Drawing for the job (mm, zero at the part's lowest x, y, z). A direction names the side the tool comes from. Give positions to 0.01 mm unless a question says otherwise; leave off trailing zeros. Order: outer loops, then holes, each group sorted by start corner. A loop starts at its lowest first (then second) coordinate and runs counter-clockwise, first axis right, second up. Notation, with made-up numbers: (4.5, 11) -> (49.5, 11) arc R23 ccw to (49.5, 41) -> close; hole circle Ø9 at (-28, 47.5). An arc over 180 degrees is marked (long way). Use one line per item in the form item = value. Start each with the question number.
1) Tool access for the marked faces 1 and 2: list every direction of +Z, -Z, +X, -X, +Y, -Y with a clear straight run to the whole face (end or side of a thin tool).
2) Cut at A-A, the plane x = 11. Give the cut face in (y, z), and give its area (4 significant figures).
3) Cut at D-D, the plane x = 17.5. Give the cut face in (y, z).
4) Cut at C-C, the plane y = 10. Give the cut face in (x, z).
5) Drop flat-ended pins along their axis: P1, Ø3, axis at x = 13, y = 34.5, coming from the -Z side; P2, Ø6.5, axis at x = 9.5, z = 11.5, coming from the -Y side; P3, Ø5, axis at y = 50.5, z = 8, coming from the +X side; P4, Ø12, axis at y = 47, z = 9.5, coming from the -X side. Give the stop position or say it passes through.
6) Probe line 1 (Y direction, x = 9.5, z = 17.25); line 2 (Y direction, x = 4.5, z = 4); line 3 (X direction, y = 72.5, z = 11.5). List the from-to ranges inside material, lowest first.
7) Cut at B-B, the plane z = 11. Give the cut face in (x, y), and give its area (4 significant figures).
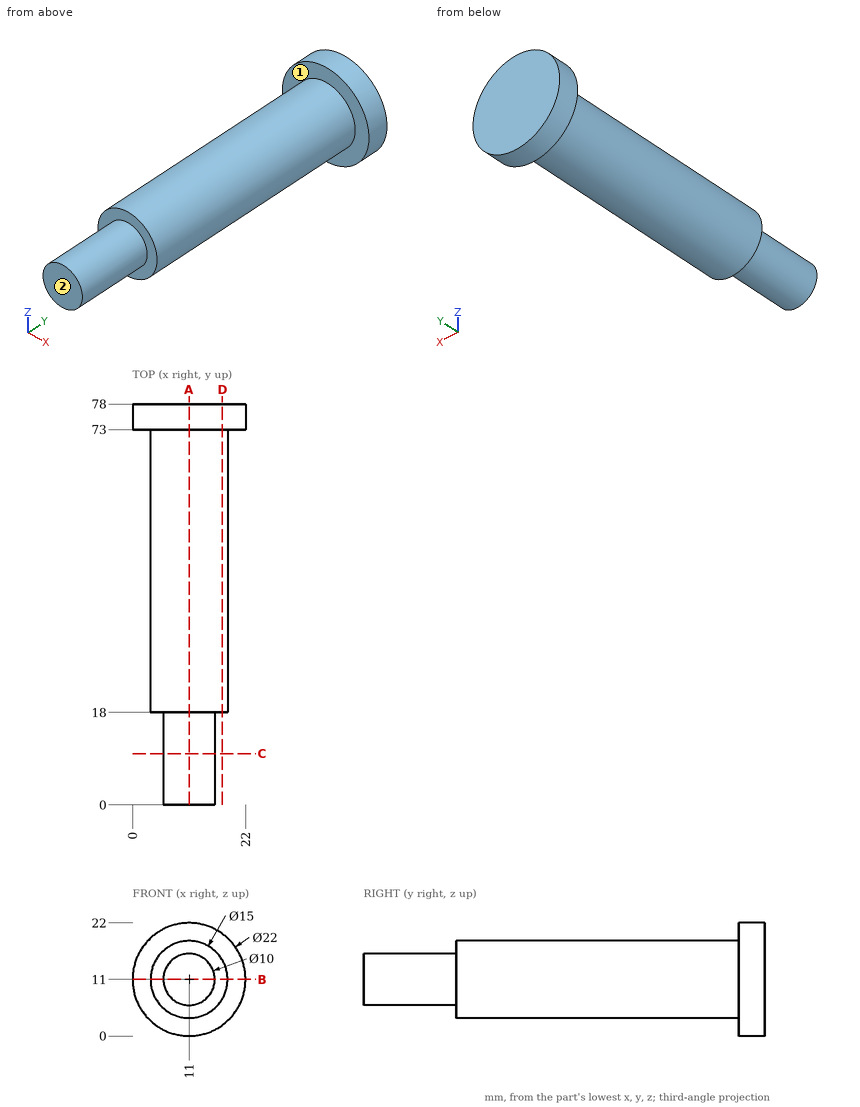
Result:
q1.face_1 = -Y
q1.face_2 = +Z, -Z, +X, -X, -Y
q2.outline = (0, 6) -> (18, 6) -> (18, 3.5) -> (73, 3.5) -> (73, 0) -> (78, 0) -> (78, 22) -> (73, 22) -> (73, 18.5) -> (18, 18.5) -> (18, 16) -> (0, 16) -> close
q2.area = 1,115 mm²
q3.outline = (18, 7.26) -> (73, 7.26) -> (73, 2.13) -> (78, 2.13) -> (78, 19.87) -> (73, 19.87) -> (73, 14.74) -> (18, 14.74) -> close
q4.outline = circle Ø10 at (11, 11)
q5.P1 = 3.52
q5.P2 = 0
q5.P3 = 18.48
q5.P4 = 3.5
q6.line_1 = 18 to 78
q6.line_2 = 73 to 78
q6.line_3 = 3.52 to 18.48
q7.outline = (0, 73) -> (3.5, 73) -> (3.5, 18) -> (6, 18) -> (6, 0) -> (16, 0) -> (16, 18) -> (18.5, 18) -> (18.5, 73) -> (22, 73) -> (22, 78) -> (0, 78) -> close
q7.area = 1,115 mm²
